Source: CAD feature listing. Evaluate the final solid. Frame: model axes, mm. A direction names the side the tool comes from. Give positions to 0.01 mm unless a question says otherwise; leave off trailing zeros. Order: outer loops, then holes, each group sorted by start corner. A loop starts at its lowest first (then second) coordinate and runs counter-clockwise, first axis right, second up. Notation, with made-up numbers: M 41,66.5 L 55,66.5 A10 ccw 55,73.5 Z; hole C 55.25,89 d1. An arc over 180 degrees is marked long. Return JSON: item names as keys, results as strings.
from build123d import *

# Parameters (mm, degrees)
SKETCH_1_W                   = 60
SKETCH_1_H                   = 120
EXTRUDE_1_DEPTH              = 2
SKETCH_2_W                   = 36
SKETCH_2_H                   = 80
CUT_EXTRUDE_1_DEPTH          = 68.201190466
SKETCH_3_W                   = 44.2
SKETCH_3_H                   = 88.2
CUT_EXTRUDE_2_DEPTH          = 1
HOLE_WIZARD_3_0_3_1_D        = 3
HOLE_WIZARD_3_0_3_1_DEPTH    = 1
FILLET_1_R                   = 3
CHAMFER_1_SIZE               = 2
HOLE_WIZARD_M3_1_D           = 3.4
HOLE_WIZARD_M3_1_CSINK_D     = 6.72
HOLE_WIZARD_M3_1_CSINK_ANGLE = 90


with BuildPart() as part:
    # 草图1 → 凸台-拉伸1 (new, symmetric)
    with BuildSketch(Plane.XY):
        Rectangle(SKETCH_1_W, SKETCH_1_H)
    extrude(amount=EXTRUDE_1_DEPTH, both=True)

    # 草图2 → 切除-拉伸1 (cut, through all)
    with BuildSketch(Plane.XY.offset(2)):
        with Locations((2, 0)):
            Rectangle(SKETCH_2_W, SKETCH_2_H)
    extrude(amount=-CUT_EXTRUDE_1_DEPTH, mode=Mode.SUBTRACT)

    # 草图3 → 切除-拉伸2 (cut)
    with BuildSketch(Plane.XY.offset(2)):
        with Locations((2, 0)):
            Rectangle(SKETCH_3_W, SKETCH_3_H)
    extrude(amount=-CUT_EXTRUDE_2_DEPTH, mode=Mode.SUBTRACT)

    # Ø3.0 (3) 直径孔1
    with Locations(Plane.XY.offset(2)):
        with Locations((-18.6, 44.1), (22.6, 44.1), (22.6, -44.1), (-18.6, -44.1)):
            Hole(HOLE_WIZARD_3_0_3_1_D / 2, depth=HOLE_WIZARD_3_0_3_1_DEPTH)

    # 圆角1
    fillet_1_edges = [part.edges().sort_by_distance(p)[0] for p in [
        (-16, -40, -0.5),
        (-16, 40, -0.5),
        (20, 40, -0.5),
        (20, -40, -0.5),
    ]]
    fillet(fillet_1_edges, radius=FILLET_1_R)

    # 倒角1
    chamfer_1_edges = [part.edges().sort_by_distance(p)[0] for p in [
        (20, 0, -2),
        (2, -40, -2),
        (-16, 0, -2),
        (19.121320344, 39.121320344, -2),
        (19.121320344, -39.121320344, -2),
        (-15.121320344, -39.121320344, -2),
        (-15.121320344, 39.121320344, -2),
        (2, 40, -2),
    ]]
    chamfer(chamfer_1_edges, length=CHAMFER_1_SIZE)

    # M3 六角凹锥坑螺钉的锥形沉头孔1 (through all)
    with Locations(Plane(origin=(0, 0, -2), x_dir=(-1, 0, 0), z_dir=(0, 0, -1))):
        with Locations((-22.5, 56), (22.5, 56), (26, 25), (26, -25), (22.5, -56), (-22.5, -56), (-26, -25), (-26, 25)):
            CounterSinkHole(HOLE_WIZARD_M3_1_D / 2, HOLE_WIZARD_M3_1_CSINK_D / 2, counter_sink_angle=HOLE_WIZARD_M3_1_CSINK_ANGLE)


solid = part.part
1. Section query A-A (y = 56). Return loops of the section in (x, z), then the cut area to 3 significant figures.
Evaluation:
{"outline": "M -30,-2 L -25.86,-2 L -24.2,-0.34 L -24.2,2 L -30,2 Z; M -20.8,-0.34 L -19.14,-2 L 19.14,-2 L 20.8,-0.34 L 20.8,2 L -20.8,2 Z; M 24.2,-0.34 L 25.86,-2 L 30,-2 L 30,2 L 24.2,2 Z", "area": "207 mm^2"}
2. Section query C-C (y = -12). Return loops of the section in (x, z), then the cut area to 3 significant figures.
Evaluation:
{"outline": "M -30,-2 L -18,-2 L -16,0 L -16,1 L -20.1,1 L -20.1,2 L -30,2 Z; M 20,0 L 22,-2 L 30,-2 L 30,2 L 24.1,2 L 24.1,1 L 20,1 Z", "area": "83.8 mm^2"}
3. Set-up query: faces 1 (the face through (-18, -7, 1)), 2 (the face through (-15.1, 39.14, 0.49)), 3 (the face through (-15.69, -39.63, -0.76)). Return all of +Z, -Z, +X, -X, +Y, -Y with unobstructed straight access to the full face (end or side cutting, diameter ignored); none if empty.
Evaluation:
{"face 1": "+Z", "face 2": "+Z, -Z", "face 3": "-Z"}
4. First-contact query: pin 1 (5.5 mm diameter, centred on x = 26, y = 25, fed in from +Z); pin 2 (4 mm diameter, centred on x = 22.5, y = 56, fed in from -Z); pin 3 (5.5 mm diameter, centred on x = 22.5, y = -56, fed in from -Z); pin 4 (3 mm diameter, centred on x = -26, y = 25, fed in from +Z). Flat tips, straight axial feed; report the tip coordinate or a pass-through.
Evaluation:
{"pin 1": "stops at z = 2", "pin 2": "stops at z = -0.64", "pin 3": "stops at z = -1.39", "pin 4": "passes through"}
5. Section query B-B (x = 2). Return loops of the section in (y, z), then the cut area to 3 significant figures.
Evaluation:
{"outline": "M -60,-2 L -42,-2 L -40,0 L -40,1 L -44.1,1 L -44.1,2 L -60,2 Z; M 40,0 L 42,-2 L 60,-2 L 60,2 L 44.1,2 L 44.1,1 L 40,1 Z", "area": "148 mm^2"}
6. Draft query along X for faces 4 (the face through (-15.63, 39.69, -0.76)), 5 (the face through (-30, -1, 0)), 6 (the face through (22.279, 57.686, 0.846)), 7 (the face through (0, -60, 0)). Return one class per face: pulls with the +X half, pulls with the -X half, needs draft (parallel to the pull), parting line crosses it, or undercut.
Evaluation:
{"face 4": "undercut", "face 5": "pulls with the -X half", "face 6": "undercut", "face 7": "needs draft"}
7. Ray query, probe 1 along Y at (x, z) = (-22.5, 0.25); probe 2 along Y at (x, z) = (26, 1.2); probe 3 along X at (y, z) = (25, 1.2). Return the intervals inside material, ascending.
Evaluation:
{"probe 1": "y = -60 to -57.7, -54.3 to 54.3, 57.7 to 60", "probe 2": "y = -60 to -26.7, -23.3 to 23.3, 26.7 to 60", "probe 3": "x = -30 to -27.7, -24.3 to -20.1, 24.1 to 24.3, 27.7 to 30"}
8. Section query D-D (y = -25). Return loops of the section in (x, z).
Evaluation:
{"outline": "M -30,-2 L -29.36,-2 L -27.7,-0.34 L -27.7,2 L -30,2 Z; M -24.3,-0.34 L -22.64,-2 L -18,-2 L -16,0 L -16,1 L -20.1,1 L -20.1,2 L -24.3,2 Z; M 20,0 L 22,-2 L 22.64,-2 L 24.3,-0.34 L 24.3,2 L 24.1,2 L 24.1,1 L 20,1 Z; M 27.7,-0.34 L 29.36,-2 L 30,-2 L 30,2 L 27.7,2 Z"}
